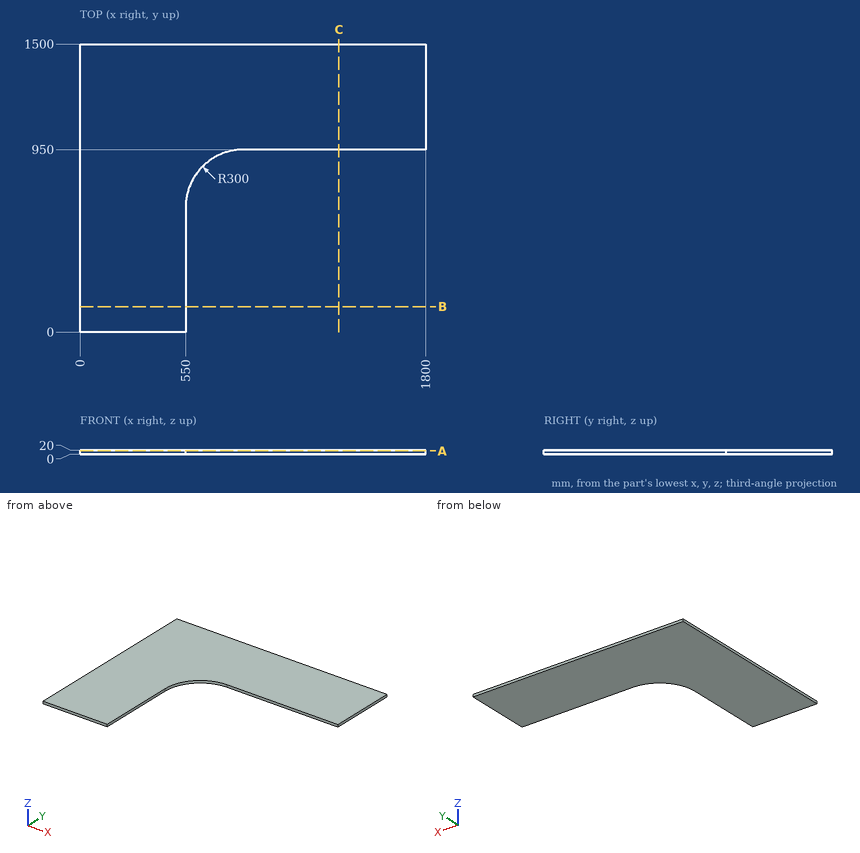
Study the drawing (mm; zero at the part's minimum x, y, z) and answer. Round coordinates to 2 decimals unless told otherwise and drop trailing zeros. Order: outer loops, then holes, each group sorted by start corner. A loop starts at its lowest first (then second) coordinate and runs counter-clockwise, first axis right, second up. Notation, with made-up numbers: (71, 3.25) -> (85, 3.25) arc R19 cw to (85, 15.25) -> close; hole circle Ø8 at (42.5, 61.5). An arc over 180 degrees is marked (long way). Answer as CSV lines item,"result". Start each with the question number.
(1) The part is cut by section B-B (y = 133). Determine the outline of the cut face in (x, z).
(2) Find the intervals of material crossed by probe 1 along X at (y, z) = (348.5, 4.75); probe 2 along Y at (x, z) = (1279, 11.5); probe 3 along X at (y, z) = (855, 6.75), in increasing order. Write a range as from..to.
(3) A flat-ended cylindrical pin translates along its axis: pin 1 Ø10 at (y, z) = (825.5, 5) entering from +X. Find the tip coordinate at first contact, or state that the pin passes through.
(4) The part is cut by section A-A (z = 16.75). Determine the outline of the cut face in (x, y).
(5) The part is cut by section C-C (x = 1348). Determine the outline of the cut face in (y, z).
Evaluation:
1,outline,"(0, 0) -> (550, 0) -> (550, 20) -> (0, 20) -> close"
2,probe 1,"0..550"
2,probe 2,"950..1500"
2,probe 3,"0..630.97"
3,pin 1,"x = 610.38"
4,outline,"(0, 0) -> (550, 0) -> (550, 650) arc R300 cw to (850, 950) -> (1800, 950) -> (1800, 1500) -> (0, 1500) -> close"
5,outline,"(950, 0) -> (1500, 0) -> (1500, 20) -> (950, 20) -> close"
